```python
from build123d import *

# Parameters (mm, degrees)
SKETCH1_W           = 10
SKETCH1_H           = 10
SKETCH1_W_2         = 9
SKETCH1_H_2         = 9
BOSS_EXTRUDE1_DEPTH = 355
SKETCH2_R           = 3
CUT_EXTRUDE1_DEPTH  = 19
SKETCH3_R           = 3
CUT_EXTRUDE2_DEPTH  = 16


with BuildPart() as part:
    # Sketch1 → Boss-Extrude1 (new body)
    with BuildSketch(Plane(origin=(0, 0, 0), x_dir=(1, 0, 0), z_dir=(0, 1, 0))):
        Rectangle(SKETCH1_W, SKETCH1_H)
        Rectangle(SKETCH1_W_2, SKETCH1_H_2, mode=Mode.SUBTRACT)
    extrude(amount=BOSS_EXTRUDE1_DEPTH)

    # Sketch2 → Cut-Extrude1 (cut)
    with BuildSketch(Plane(origin=(0, 0, -5), x_dir=(-1, 0, 0), z_dir=(0, 0, -1))):
        with Locations((0, 5)):
            Circle(SKETCH2_R)
    extrude(amount=-CUT_EXTRUDE1_DEPTH, mode=Mode.SUBTRACT)

    # Sketch3 → Cut-Extrude2 (cut)
    with BuildSketch(Plane(origin=(0, 0, -5), x_dir=(-1, 0, 0), z_dir=(0, 0, -1))):
        with Locations((0, 350)):
            Circle(SKETCH3_R)
    extrude(amount=-CUT_EXTRUDE2_DEPTH, mode=Mode.SUBTRACT)


solid = part.part
```
Build history of the part. All positions in model axes, mm. A direction names the side the tool comes from. Round coordinates to 2 decimals unless told otherwise and drop trailing zeros. Write each loop counter-clockwise with the first axis right and the second up, starting at its lowest first coordinate (ties: lowest second). Pieces come first, ordered by that corner, then holes.
1) Drill centre lines: probe 1 along Y at (x, z) = (0, 4.85); probe 2 along X at (y, z) = (36, -3.25). Where is each one in solid material? Low to high.
2) Mould opens along X. For faces 3 (the flat face through (0, 175, 4.5)), 4 (the flat face through (-0.4, 355, 4.8)), 5 (the flat face through (-5, 175, 0)) say: +X half, -X half, draft (parallel to the pull), parting line (faces both ways), or undercut.
3) Band-saw the part on A-A, the plane y = 350. List the corners of the cut face in (x, z).
4) Band-saw the part on C-C, the plane y = 219.5. List the corners of the cut face in (x, z).
5) Band-saw the part on B-B, the plane x = 0. List the corners of the cut face in (y, z).
6) 3-axis set-ups, long thin cutter, end or side, ignore diameter. For faces 1 (the flat face through (0, 175, -4.5)), 2 (the cylindrical face through (0.391, 352.974, -4.754)): which of +Z, -Z, +X, -X, +Y, -Y reach the whole face in a straight line?
Ans:
1. probe 1: y = 0 to 2, 8 to 347, 353 to 355
1. probe 2: x = -5 to -4.5, 4.5 to 5
2. face 3: undercut
2. face 4: draft
2. face 5: -X half
3. outline: (-5, -5) - (-3, -5) - (-3, -4.5) - (-4.5, -4.5) - (-4.5, 4.5) - (-3, 4.5) - (-3, 5) - (-5, 5) - close; (3, -5) - (5, -5) - (5, 5) - (3, 5) - (3, 4.5) - (4.5, 4.5) - (4.5, -4.5) - (3, -4.5) - close
4. outline: (-5, -5) - (5, -5) - (5, 5) - (-5, 5) - close; hole (-4.5, -4.5) - (4.5, -4.5) - (4.5, 4.5) - (-4.5, 4.5) - close
5. outline: (0, -5) - (2, -5) - (2, -4.5) - (0, -4.5) - close; (0, 4.5) - (2, 4.5) - (2, 5) - (0, 5) - close; (8, -5) - (347, -5) - (347, -4.5) - (8, -4.5) - close; (8, 4.5) - (347, 4.5) - (347, 5) - (8, 5) - close; (353, -5) - (355, -5) - (355, -4.5) - (353, -4.5) - close; (353, 4.5) - (355, 4.5) - (355, 5) - (353, 5) - close
6. face 1: +Y, -Y
6. face 2: +Z, -Z
